from build123d import *

# Parameters (mm, degrees)
SKETCH1_R           = 8
SKETCH1_R_2         = 7
BOSS_EXTRUDE1_DEPTH = 13
CUT_EXTRUDE1_START  = -1
CUT_EXTRUDE1_DEPTH  = 1
CHAMFER2_SIZE       = 0.5
SKETCH3_R           = 3.25
CUT_EXTRUDE2_DEPTH  = 17


with BuildPart() as part:
    # Sketch1 → Boss-Extrude1 (new body)
    with BuildSketch(Plane.XY):
        with BuildLine():
            Line((0, 5), (0, 25))
            Line((0, 25), (63, 25))
            Line((63, 25), (68, -34.543411946))
            Line((68, -34.543411946), (33.385133941, -34.543411946))
            ThreePointArc((33.385133941, -34.543411946), (30.752722356, -33.794342344), (28.909054571, -31.771575646))
            Line((28.909054571, -31.771575646), (14.473169684, -2.7718363))
            ThreePointArc((14.473169684, -2.7718363), (12.629501898, -0.749069602), (9.997090314, 0))
            Line((9.997090314, 0), (5, 0))
            ThreePointArc((5, 0), (1.464466094, 1.464466094), (0, 5))
        make_face()
        with Locations(Location((21.645133941, 13, 0), (0, 0, 180))):
            Circle(SKETCH1_R, mode=Mode.SUBTRACT)
        with Locations(Location((33.385133941, -12.47, 0), (0, 0, 180))):
            Circle(SKETCH1_R_2, mode=Mode.SUBTRACT)
    extrude(amount=BOSS_EXTRUDE1_DEPTH)

    # Sketch2 → Cut-Extrude1 (cut)
    with BuildSketch(Plane.XY.offset(13).offset(CUT_EXTRUDE1_START)):
        with BuildLine():
            Line((48, 25), (58, -34.543411946))
            Line((58, -34.543411946), (33.385133941, -34.543411946))
            ThreePointArc((33.385133941, -34.543411946), (30.752722356, -33.794342344), (28.909054571, -31.771575646))
            Line((28.909054571, -31.771575646), (14.473169684, -2.7718363))
            ThreePointArc((14.473169684, -2.7718363), (12.629501898, -0.749069602), (9.997090314, 0))
            Line((9.997090314, 0), (5, 0))
            ThreePointArc((5, 0), (1.464466094, 1.464466094), (0, 5))
            Line((0, 5), (0, 25))
            Line((0, 25), (48, 25))
        make_face()
    extrude(amount=CUT_EXTRUDE1_DEPTH, mode=Mode.SUBTRACT)

    # Chamfer2
    chamfer2_edges = [part.edges().sort_by_distance(p)[0] for p in [
        (29.645133941, 13, 0),
        (40.385133941, -12.47, 0),
        (29.645133941, 13, 12),
        (40.385133941, -12.47, 12),
    ]]
    chamfer(chamfer2_edges, length=CHAMFER2_SIZE)

    # Sketch3 → Cut-Extrude2 (cut)
    with BuildSketch(Plane.ZY):
        with Locations((6, 13)):
            Circle(SKETCH3_R)
    extrude(amount=-CUT_EXTRUDE2_DEPTH, mode=Mode.SUBTRACT)


solid = part.part
Input: part model. Units: mm. Frame: model coordinates. A direction names the side the tool comes from. Round coordinates to 2 decimals unless told otherwise and drop trailing zeros. Order: outer loops, then holes, each group sorted by start corner. A loop starts at its lowest first (then second) coordinate and runs counter-clockwise, first axis right, second up. Notation, with made-up numbers: (83.25, 62.25) - (113.25, 62.25) arc R15 cw to (113.25, 83.25) - close; hole circle Ø11 at (48, -26). An arc over 180 degrees is marked (long way). Use a Markdown table: item, result.
1. Section B-B on z = 10.5. Return the cut outline in (x, y).
Evaluation:
| item | result |
|---|---|
| outline | (0, 5) arc R5 ccw to (5, 0) - (10, 0) arc R5 cw to (14.47, -2.77) - (28.91, -31.77) arc R5 ccw to (33.39, -34.54) - (68, -34.54) - (63, 25) - (0, 25) - close; hole circle Ø16 at (21.65, 13); hole circle Ø14 at (33.39, -12.47) |
2. Material intervals for probe 1 along Y at (x, z) = (28.5, 10.75); probe 2 along Y at (x, z) = (33, 7); probe 3 along Z at (x, y) = (41.5, -5.5), sorted ascending.
Evaluation:
| item | result |
|---|---|
| probe 1 | -30.95 to -17.48, -7.46 to 8.88, 17.12 to 25 |
| probe 2 | -34.53 to -19.46, -5.48 to 25 |
| probe 3 | 0 to 12 |
3. Access query for faces 4 (the face through (29, -4, 12)), 5 (the face through (40.38, -12.78, 5.92)), 6 (the face through (7.07, 15.74, 7.75)), 7 (the face through (31, 25, 6)), 8 (the face through (8, 0, 6)). Directions: +Z, -Z, +X, -X, +Y, -Y. A direction counts if a zero-diameter tool reaches every point of the face in a straight line with its end or side. Return the directions, or none.
Evaluation:
| item | result |
|---|---|
| face 4 | +Z, -X, -Y |
| face 5 | +Z, -Z |
| face 6 | -X |
| face 7 | +Z, -Z, +X, -X, +Y |
| face 8 | +Z, -Z, -X, -Y |
4. First-contact query: pin 1 (2.5 mm diameter, centred on x = 6.5, z = 8, fed in from -Y); pin 2 (1 mm diameter, centred on x = 11, z = 9, fed in from -Y); pin 3 (3 mm diameter, centred on y = -3.5, z = 2, fed in from +X); pin 4 (12.5 mm diameter, centred on x = 33.39, y = -12.47, fed in from -Z). Flat tips, straight axial feed; report the tip coordinate or a pass-through.
Evaluation:
| item | result |
|---|---|
| pin 1 | y = 0 |
| pin 2 | y = -0.23 |
| pin 3 | x = 65.52 |
| pin 4 | through |
5. Section A-A on z = 6. Return the cut outline in (x, y), then the cut area to 3 significant figures.
Evaluation:
| item | result |
|---|---|
| outline | (0, 5) arc R5 ccw to (5, 0) - (10, 0) arc R5 cw to (14.47, -2.77) - (28.91, -31.77) arc R5 ccw to (33.39, -34.54) - (68, -34.54) - (63, 25) - (0, 25) - (0, 16.25) - (14.34, 16.25) arc R8 cw (long way) to (14.34, 9.75) - (0, 9.75) - close; hole circle Ø14 at (33.39, -12.47) |
| area | 2,700 mm^2 |
6. Section D-D on y = 13. Return the cut outline in (x, z), then the cut area to 3 significant figures.
Evaluation:
| item | result |
|---|---|
| outline | (0, 0) - (13.15, 0) - (13.65, 0.5) - (13.65, 2.75) - (0, 2.75) - close; (0, 9.25) - (13.65, 9.25) - (13.65, 11.5) - (13.15, 12) - (0, 12) - close; (29.65, 0.5) - (30.15, 0) - (64.01, 0) - (64.01, 13) - (50.02, 13) - (50.02, 12) - (30.15, 12) - (29.65, 11.5) - close |
| area | 501 mm^2 |
7. Section C-C on y = -12.47. Return the cut outline in (x, z), then the cut area to 4 significant figures.
Evaluation:
| item | result |
|---|---|
| outline | (19.3, 0) - (25.89, 0) - (26.39, 0.5) - (26.39, 11.5) - (25.89, 12) - (19.3, 12) - close; (40.39, 0.5) - (40.89, 0) - (66.15, 0) - (66.15, 13) - (54.29, 13) - (54.29, 12) - (40.89, 12) - (40.39, 11.5) - close |
| area | 405.5 mm^2 |
8. Mould query, pull axis X, two halves, no side actions, for faces 1 (the face through (0, 17, 6)), 2 (the face through (58, -4, 13)), 3 (the face through (29.637, 12.648, 5.923)). Classes: +X half, -X half, draft (parallel to the pull), parting line (faces both ways), or undercut.
Evaluation:
| item | result |
|---|---|
| face 1 | -X half |
| face 2 | draft |
| face 3 | undercut |
